```python
from build123d import *

# Parameters (mm, degrees)
SKETCH1_W                                            = 28
SKETCH1_H                                            = 26
BOSS_EXTRUDE1_DEPTH                                  = 470
HOLE_SIZE_PER_SOCKET_HEAD_CAP_SCREW_TYPE_D           = 9
HOLE_SIZE_PER_SOCKET_HEAD_CAP_SCREW_TYPE_CBORE_D     = 15
HOLE_SIZE_PER_SOCKET_HEAD_CAP_SCREW_TYPE_CBORE_DEPTH = 9
LPATTERN1_COUNT                                      = 6
LPATTERN1_PITCH                                      = 80


with BuildPart() as part:
    # Sketch1 → Boss-Extrude1 (new body)
    with BuildSketch(Plane.XY):
        Rectangle(SKETCH1_W, SKETCH1_H)
    extrude(amount=-BOSS_EXTRUDE1_DEPTH)

    # Hole size per socket head cap screw type1 (through all)
    with Locations(Plane(origin=(0, 13, 0), x_dir=(-1, 0, 0), z_dir=(0, 1, 0))):
        with Locations((0, -35)):
            hole_size_per_socket_head_cap_screw_type = CounterBoreHole(HOLE_SIZE_PER_SOCKET_HEAD_CAP_SCREW_TYPE_D / 2, HOLE_SIZE_PER_SOCKET_HEAD_CAP_SCREW_TYPE_CBORE_D / 2, HOLE_SIZE_PER_SOCKET_HEAD_CAP_SCREW_TYPE_CBORE_DEPTH)

    # LPattern1: Hole size per socket head cap screw type1 ×6
    with Locations(*[(0, 0, -i * LPATTERN1_PITCH) for i in range(1, LPATTERN1_COUNT)]):
        add(hole_size_per_socket_head_cap_screw_type, mode=Mode.SUBTRACT)


solid = part.part
```
Geometry check sheet. Reference: the model listing, model coordinates, mm. A direction names the side the tool comes from. Coordinates: 2 decimals unless noted, no trailing zeros. Write each loop counter-clockwise with the first axis right and the second up, starting at its lowest first coordinate (ties: lowest second). Pieces come first, ordered by that corner, then holes. Notation, with made-up numbers: M 29,-32.5 L 53,-32.5 A32 ccw 53,-4.5 Z; hole C 27,0.25 d3. An arc over 180 degrees is marked long. One line per item, written item: value. Start each with the question number.
(1) Sectioned sample at B-B, the plane y = 0. Enter the section's corners in (x, z), and give its area (3 significant figures).
(2) Sectioned sample at A-A, the plane z = -275. Enter the section's corners in (x, y).
(3) Release check for a two-part mould opening along Z. For faces 3 (the face through (-14, 0, -232)), 4 (the face through (1.63, 8.56, -362.32)), 5 (the face through (0, 0, -470)) record: released by +Z, released by -Z, zero draft, split by the parting line, or undercut.
(4) Tool access check on faces 1 (the face through (1.63, 8.56, -282.32)), 2 (the face through (0, 0, 0)). Record the directions out of +Z, -Z, +X, -X, +Y, -Y that give a thin tool (end or side, any length) a straight path to the whole face; none if there is none.
(5) Scan lines: line 1 along X through (y, z) = (0, -275); line 2 along X through (y, z) = (8, -435); line 3 along Y through (x, z) = (-4.5, -351). Record each from-to range of solid material in increasing order. Write a range as [from, to].
(6) Sectioned sample at C-C, the plane x = 0. State how many separate pieces and enclosed holes the cut face has, and give its area (3 significant figures).
(7) Depth check by flat-ended pin: pin 1 (10.5 mm diameter, centred on x = 0, z = -115, fed in from +Y). Enter the tip coordinate at first touch or a pass-through.
Filled sheet:
1. outline: M -14,-470 L 14,-470 L 14,0 L -14,0 Z; hole C 0,-435 d9; hole C 0,-355 d9; hole C 0,-275 d9; hole C 0,-195 d9; hole C 0,-115 d9; hole C 0,-35 d9
1. area: 12,800 mm²
2. outline: M -14,-13 L -4.5,-13 L -4.5,4 L -7.5,4 L -7.5,13 L -14,13 Z; M 4.5,-13 L 14,-13 L 14,13 L 7.5,13 L 7.5,4 L 4.5,4 Z
3. face 3: zero draft
3. face 4: undercut
3. face 5: released by -Z
4. face 1: +Y
4. face 2: +Z, +X, -X, +Y, -Y
5. line 1: [-14, -4.5], [4.5, 14]
5. line 2: [-14, -7.5], [7.5, 14]
5. line 3: [-13, 4]
6. separate pieces: 7
6. enclosed holes: 0
6. area: 10,500 mm²
7. pin 1: y = 4
